from build123d import *

# Parameters (mm, degrees)
CHAMFERED_END_WALL_DEPTH = 10
BACK_WALL_SKETCH_W       = 10
BACK_WALL_SKETCH_H       = 40
BACK_WALL_DEPTH          = 40
BASE_PLATE_SKETCH_W      = 60
BASE_PLATE_SKETCH_H      = 10
BASE_PLATE_DEPTH         = 40
BASE_SLOT_SKETCH_W       = 40
BASE_SLOT_SKETCH_H       = 20
BASE_SLOT_40X20_DEPTH    = 10


with BuildPart() as part:
    # End Wall Profile Sketch → Chamfered End Wall (new body)
    with BuildSketch(Plane.XY):
        Polygon((0, 0), (0, 40), (40, 40), (70, 20), (70, 0), align=None)
    extrude(amount=CHAMFERED_END_WALL_DEPTH)

    # Back Wall Sketch → Back Wall (add)
    with BuildSketch(Plane.XY.offset(10)):
        with Locations((5, 20)):
            Rectangle(BACK_WALL_SKETCH_W, BACK_WALL_SKETCH_H)
    extrude(amount=BACK_WALL_DEPTH)

    # Base Plate Sketch → Base Plate (add)
    with BuildSketch(Plane.XY.offset(10)):
        with Locations((40, 5)):
            Rectangle(BASE_PLATE_SKETCH_W, BASE_PLATE_SKETCH_H)
    extrude(amount=BASE_PLATE_DEPTH)

    # Base Slot Sketch → Base Slot 40x20 (cut)
    with BuildSketch(Plane(origin=(0, 10, 0), x_dir=(1, 0, 0), z_dir=(0, 1, 0))):
        with Locations((40, -30)):
            Rectangle(BASE_SLOT_SKETCH_W, BASE_SLOT_SKETCH_H)
    extrude(amount=-BASE_SLOT_40X20_DEPTH, mode=Mode.SUBTRACT)


solid = part.part
Design review of the part built by this model. Coordinates are the model's own, in mm. A direction names the side the tool comes from. Coordinates: 2 decimals unless noted, no trailing zeros. Write each loop counter-clockwise with the first axis right and the second up, starting at its lowest first coordinate (ties: lowest second). Pieces come first, ordered by that corner, then holes. Notation, with made-up numbers: (82.25, 16) -> (124.25, 16) arc R15 cw to (124.25, 20) -> close; hole circle Ø7 at (-27.5, -14). An arc over 180 degrees is marked (long way). Write each question's results on one line, items separated by ' | '. Start each with the question number.
(1) Take a section at B-B on y = 5. Write out the cut boundary in (x, z), and give its area (3 significant figures).
(2) Take a section at A-A on x = 49. Write out the cut boundary in (y, z).
(3) Clearance check with flat-ended pins moving along their axes: P1, Ø9, axis at x = 45.5, y = 22, coming from the +Z side; P2, Ø2, axis at y = 34, z = 27.5, coming from the +X side; P3, Ø4, axis at x = 21.5, z = 34, coming from the +Y side. State where each tip first meets the part, or that it passes through.
(4) For line 1 along X through (y, z) = (8, 39); line 2 along Z through (x, y) = (23.5, 6.5); line 3 along Z through (x, y) = (43, 31.5), list the stretches that pass through material, from the lowest coordinate up. Write a range as from..to.
(5) Tool access review of faces 5 (the face through (10, 25, 30)), 6 (the face through (20, 5, 30)), 7 (the face through (6, 40, 14)): name each direction out of +Z, -Z, +X, -X, +Y, -Y from which nothing blocks a thin tool from reaching the whole face with its end or side.
(6) Take a section at C-C on z = 23.5. Write out the cut boundary in (x, y).
(7) Take a section at D-D on x = 61. Write out the cut boundary in (y, z).
(8) The part is to be moulded in two halves that separate along Z. For faces 1 (the face through (40, 5, 20)), 2 (the face through (35, 20, 0)), 3 (the face through (34, 25, 10)), 4 (the face through (35, 0, 19)), say which applies: pulls with the +Z half, pulls with the -Z half, needs draft (parallel to the pull), parting line crosses it, or undercut.
Results found:
1) outline: (0, 0) -> (70, 0) -> (70, 50) -> (0, 50) -> close; hole (20, 20) -> (60, 20) -> (60, 40) -> (20, 40) -> close | area: 2,700 mm2
2) outline: (0, 0) -> (34, 0) -> (34, 10) -> (10, 10) -> (10, 20) -> (0, 20) -> close; (0, 40) -> (10, 40) -> (10, 50) -> (0, 50) -> close
3) P1: stops at z = 10 | P2: stops at x = 10 | P3: stops at y = 10
4) line 1: x = 0..20, 60..70 | line 2: z = 0..20, 40..50 | line 3: z = 0..10
5) face 5: +Z, +X, +Y | face 6: +Y, -Y | face 7: +Z, -Z, +X, -X, +Y
6) outline: (0, 0) -> (20, 0) -> (20, 10) -> (10, 10) -> (10, 40) -> (0, 40) -> close; (60, 0) -> (70, 0) -> (70, 10) -> (60, 10) -> close
7) outline: (0, 0) -> (26, 0) -> (26, 10) -> (10, 10) -> (10, 50) -> (0, 50) -> close
8) face 1: undercut | face 2: pulls with the -Z half | face 3: pulls with the +Z half | face 4: needs draft
